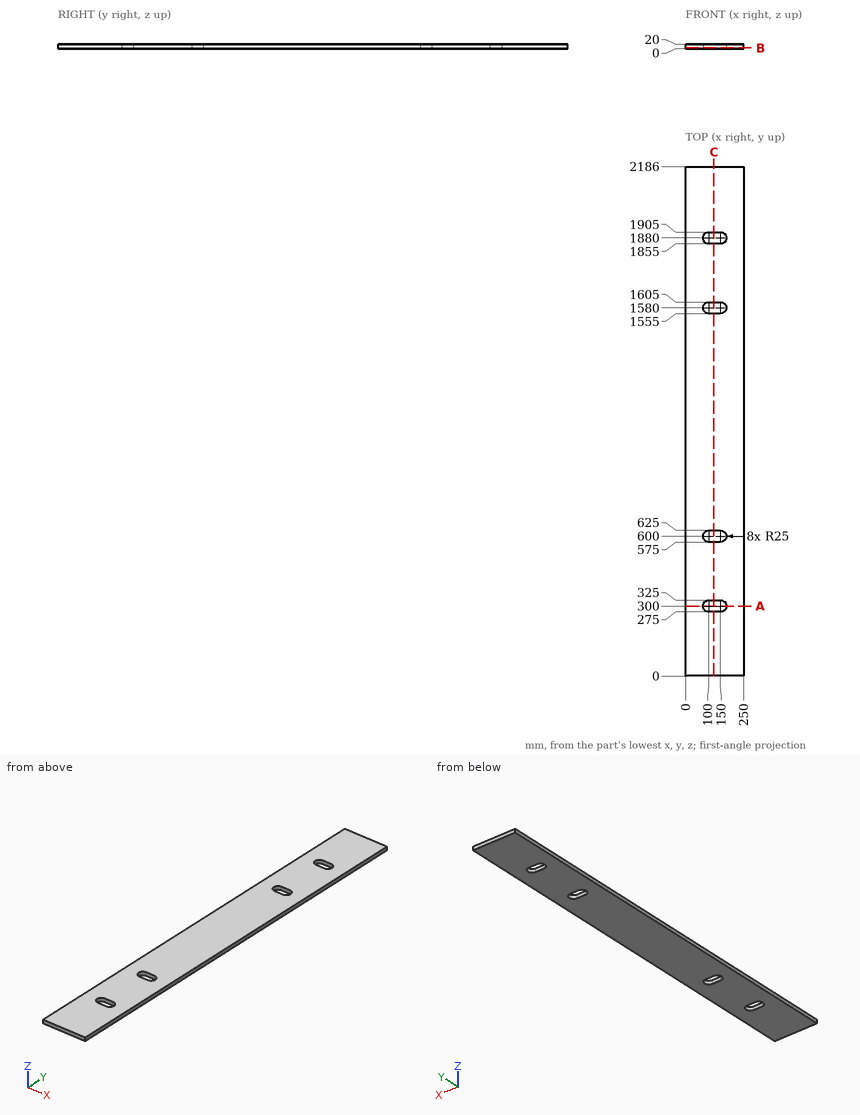
Can you work these out from the drawing? Everything is in mm from the part's minimum corner. Give positions to 0.01 mm unless a question says otherwise; leave off trailing zeros. Order: outer loops, then holes, each group sorted by start corner. A loop starts at its lowest first (then second) coordinate and runs counter-clockwise, first axis right, second up. Notation, with made-up numbers: M 81,71 L 92,71 A22 cw 92,94 Z; hole C 34.25,8.5 d2. An arc over 180 degrees is marked long. Use a Markdown table: item, result. Add a question column.
1. Suppose I cut it at B-B (z = 3.5). List the corners of the cut face in (x, y) for me.
2. Suppose I cut it at C-C (x = 122). List the corners of the cut face in (y, z) for me, and give its area (3 significant figures).
3. Suppose I cut it at A-A (y = 300). List the corners of the cut face in (x, z) for me, and give its area (3 significant figures).
4. I need wall thicknesses on probe 1 along Y at (x, z) = (134.5, 4.5); probe 2 along Y at (x, z) = (153, 17). Which ranges of each line are inside material? Lowest first, please. Write a range as from..to.
Results list:
| question | item | result |
|---|---|---|
| 1 | outline | M 0,0 L 250,0 L 250,2186 L 0,2186 Z; hole M 100,275 L 150,275 A25 ccw 150,325 L 100,325 A25 ccw Z; hole M 100,575 L 150,575 A25 ccw 150,625 L 100,625 A25 ccw Z; hole M 100,1555 L 150,1555 A25 ccw 150,1605 L 100,1605 A25 ccw Z; hole M 100,1855 L 150,1855 A25 ccw 150,1905 L 100,1905 A25 ccw Z |
| 2 | outline | M 0,0 L 275,0 L 275,20 L 0,20 Z; M 325,0 L 575,0 L 575,20 L 325,20 Z; M 625,0 L 1555,0 L 1555,20 L 625,20 Z; M 1605,0 L 1855,0 L 1855,20 L 1605,20 Z; M 1905,0 L 2186,0 L 2186,20 L 1905,20 Z |
| 2 | area | 39,700 mm² |
| 3 | outline | M 0,0 L 75,0 L 75,20 L 0,20 Z; M 175,0 L 250,0 L 250,20 L 175,20 Z |
| 3 | area | 3,000 mm² |
| 4 | probe 1 | y = 0..275, 325..575, 625..1555, 1605..1855, 1905..2186 |
| 4 | probe 2 | y = 0..275.18, 324.82..575.18, 624.82..1555.18, 1604.82..1855.18, 1904.82..2186 |
